from build123d import *

# Parameters (mm, degrees)
SKETCH_1_W                   = 317
SKETCH_1_H                   = 25
EXTRUDE_1_DEPTH              = 8
HOLE_WIZARD_M5_1_D           = 5.5
HOLE_WIZARD_M5_1_CBORE_D     = 10
HOLE_WIZARD_M5_1_CBORE_DEPTH = 5.4
SKETCH_4_R                   = 2.5
CUT_EXTRUDE_1_DEPTH          = 160.193278753
SKETCH_7_W                   = 277
SKETCH_7_H                   = 4
EXTRUDE_2_DEPTH              = 8
HOLE_WIZARD_M4_1_D           = 4.5
HOLE_WIZARD_M4_1_CBORE_D     = 8
HOLE_WIZARD_M4_1_CBORE_DEPTH = 4.4
CHAMFER_3_SIZE               = 1


with BuildPart() as part:
    # 草图1 → 凸台-拉伸1 (new body)
    with BuildSketch(Plane(origin=(0, 0, 0), x_dir=(1, 0, 0), z_dir=(0, 1, 0))):
        Rectangle(SKETCH_1_W, SKETCH_1_H)
    extrude(amount=EXTRUDE_1_DEPTH)

    # M5 六角凹头螺钉的柱形沉头孔1 (through all)
    with Locations(Plane(origin=(0, 8, 0), x_dir=(1, 0, 0), z_dir=(0, 1, 0))):
        with Locations((-152.5, -6.5), (152.5, -6.5)):
            CounterBoreHole(HOLE_WIZARD_M5_1_D / 2, HOLE_WIZARD_M5_1_CBORE_D / 2, HOLE_WIZARD_M5_1_CBORE_DEPTH)

    # 草图4 → 切除-拉伸1 (cut, through all)
    with BuildSketch(Plane(origin=(0, 8, 0), x_dir=(1, 0, 0), z_dir=(0, 1, 0))):
        with Locations(Location((-152.5, 2, 0), (0, 0, 270))):
            Circle(SKETCH_4_R)
        with Locations(Location((152.5, 2, 0), (0, 0, 270))):
            Circle(SKETCH_4_R)
    extrude(amount=-CUT_EXTRUDE_1_DEPTH, mode=Mode.SUBTRACT)

    # 草图7 → 凸台-拉伸2 (add)
    with BuildSketch(Plane.XZ):
        with Locations((0, -14.5)):
            Rectangle(SKETCH_7_W, SKETCH_7_H)
    extrude(amount=-EXTRUDE_2_DEPTH)

    # M4 六角凹头螺钉的柱形沉头孔1 (through all)
    with Locations(Plane(origin=(0, 0, 0), x_dir=(-1, 0, 0), z_dir=(0, -1, 0))):
        with Locations((-120, 11), (-40, 11), (40, 11), (120, 11)):
            CounterBoreHole(HOLE_WIZARD_M4_1_D / 2, HOLE_WIZARD_M4_1_CBORE_D / 2, HOLE_WIZARD_M4_1_CBORE_DEPTH)

    # 倒角3
    chamfer_3_edges = [part.edges().sort_by_distance(p)[0] for p in [
        (-158.5, 4, -12.5),
        (-158.5, 4, 12.5),
        (158.5, 4, -12.5),
        (158.5, 4, 12.5),
    ]]
    chamfer(chamfer_3_edges, length=CHAMFER_3_SIZE)


solid = part.part
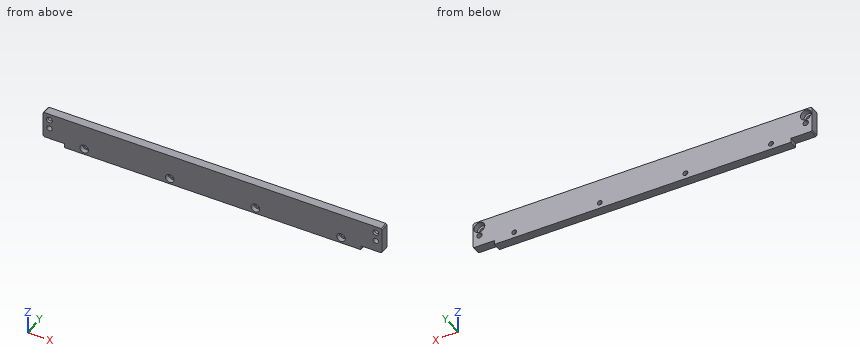
The model under review builds one solid part; all positions refer to its coordinate system, in mm. Give positions to 0.01 mm unless a question says otherwise; leave off trailing zeros. Loops run counter-clockwise (first coordinate to the right, second up) from the corner with the lowest first, then second, coordinate; pieces in that order, holes last. Notation, with made-up numbers: (-22, -14) -> (0, -14) arc R18 ccw to (0, 16) -> close; hole circle Ø8 at (7.5, 14.5). An arc over 180 degrees is marked (long way). Answer as a JSON object with one key per item and string values. Group by question number.
Q1. Wall thickness on line 1 along Z through (x, y) = (152.5, 4.25); line 2 along X through (y, z) = (6.5, -11); line 3 along X through (y, z) = (5.75, -2): over which ranges is each line inside the solid? List them lowest first.
Q2. Insertion check: pin 1 (4.5 mm diameter, centred on x = 152.5, z = -2, fed in from +Y); pin 2 (3 mm diameter, centred on y = 4, z = -15.5, fed in from +X); pin 3 (7 mm diameter, centred on x = 120, z = -11, fed in from -Y); pin 4 (7 mm diameter, centred on x = -152.5, z = 6.5, fed in from +Y). Each pin has a flat end and moves straight along its axis. Give the tip position at first contact, or say it passes through.
Q3. Take a section at A-A (z = 6.5). Write out the cut boundary in (x, y).
Answer below:
{
 "1": {"line 1": "z = -12.5 to -4.5, 0.5 to 1.5, 11.5 to 12.5", "line 2": "x = -158.5 to -122.25, -117.75 to -42.25, -37.75 to 37.75, 42.25 to 117.75, 122.25 to 158.5", "line 3": "x = -158.5 to -155, -150 to 150, 155 to 158.5"},
 "2": {"pin 1": "passes through", "pin 2": "stops at x = 138.5", "pin 3": "stops at y = 4.4", "pin 4": "stops at y = 2.6"},
 "3": {"outline": "(-158.5, 0) -> (-155.25, 0) -> (-155.25, 2.6) -> (-157.5, 2.6) -> (-157.5, 8) -> (-158.5, 8) -> close; (-149.75, 0) -> (149.75, 0) -> (149.75, 2.6) -> (147.5, 2.6) -> (147.5, 8) -> (-147.5, 8) -> (-147.5, 2.6) -> (-149.75, 2.6) -> close; (155.25, 0) -> (158.5, 0) -> (158.5, 8) -> (157.5, 8) -> (157.5, 2.6) -> (155.25, 2.6) -> close"}
}
